CAD build for the part. Positions are in the model's coordinates, mm. Give positions to 0.01 mm unless a question says otherwise; leave off trailing zeros. Write each loop counter-clockwise with the first axis right and the second up, starting at its lowest first coordinate (ties: lowest second). Pieces come first, ordered by that corner, then holes. Notation, with made-up numbers: M 7.25,86.5 L 20.25,86.5 A18 cw 20.25,95.5 Z; hole C 78.25,68 d1. An arc over 180 degrees is marked long. One line per question, with ' | ' between items. Start each with the question number.
1. Cut at B-B, the plane y = 526. Write the cut outline in (x, z), then the cut area to 3 significant figures.
2. Cut at A-A, the plane z = 1. Write the cut outline in (x, y), then the cut area to 3 significant figures.
3. Wall check: L1, parallel to Y at x = 0, z = 4.4; L2, parallel to Z at x = 0.75, y = 733.5; L3, parallel to X at y = 132, z = -2. Give the ranges that are in metal, low to high.
4. Flat gauge pin, fed straight in: pin 1 (6 mm diameter, centred on x = 0, y = 1538.3, fed in from -Z). Where does the tip first touch, or does it go through?
```python
from build123d import *

# Parameters (mm, degrees)
SKETCH_2_W                = 20
SKETCH_2_H                = 10
SKETCH_2_W_2              = 18
SKETCH_2_H_2              = 8
EXTRUDE_1_DEPTH           = 1546.3
HOLE_WIZARD_1_D           = 5.5
HOLE_WIZARD_1_CBORE_D     = 10
HOLE_WIZARD_1_CBORE_DEPTH = 5.7


with BuildPart() as part:
    # 草图2 → 凸台-拉伸1 (new body)
    with BuildSketch(Plane(origin=(0, 0, 0), x_dir=(1, 0, 0), z_dir=(0, 1, 0))):
        Rectangle(SKETCH_2_W, SKETCH_2_H)
        Rectangle(SKETCH_2_W_2, SKETCH_2_H_2, mode=Mode.SUBTRACT)
    extrude(amount=EXTRUDE_1_DEPTH)

    # 打孔尺寸(%根据)内六角圆柱头螺钉的类型1 (through all)
    with Locations(Plane(origin=(0, 0, -5), x_dir=(-1, 0, 0), z_dir=(0, 0, -1))):
        with Locations((0, 1538.3), (0, 8)):
            CounterBoreHole(HOLE_WIZARD_1_D / 2, HOLE_WIZARD_1_CBORE_D / 2, HOLE_WIZARD_1_CBORE_DEPTH)


solid = part.part
```
Here are the results:
1) outline: M -10,-5 L 10,-5 L 10,5 L -10,5 Z; hole M -9,-4 L 9,-4 L 9,4 L -9,4 Z | area: 56.0 mm^2
2) outline: M -10,0 L -9,0 L -9,1546.3 L -10,1546.3 Z; M 9,0 L 10,0 L 10,1546.3 L 9,1546.3 Z | area: 3,090 mm^2
3) L1: 0 to 5.25, 10.75 to 1535.55, 1541.05 to 1546.3 | L2: -5 to -4, 4 to 5 | L3: -10 to -9, 9 to 10
4) pin 1: z = 4
